The listing builds one solid part. Answer for the finished solid, in the listing's coordinates (mm). A direction names the side the tool comes from. Round coordinates to 2 decimals unless told otherwise and drop trailing zeros. Loops run counter-clockwise (first coordinate to the right, second up) from the corner with the lowest first, then second, coordinate; pieces in that order, holes last. Notation, with made-up numbers: (8.5, -23) - (38.5, -23) arc R32 cw to (38.5, 15) - close; hole circle Ø11 at (-31.5, 44). An arc over 180 degrees is marked (long way). One line per item, written item: value.
```python
from build123d import *

# Parameters (mm, degrees)
FLANGE_SKETCH_R              = 30
FRONT_FLANGE_60_DEPTH        = 16
FRONT_MAIN_JOURNAL_PROFILE_W = 15
FRONT_MAIN_JOURNAL_PROFILE_H = 62
CRANK_WEB_1_DEPTH            = 22
CRANKPIN_1_PROFILE_W         = 20
CRANKPIN_1_PROFILE_H         = 35
CRANK_WEB_2_DEPTH            = 25
MAIN_JOURNAL_2_PROFILE_W     = 22.5
MAIN_JOURNAL_2_PROFILE_H     = 35
CRANK_WEB_3_DEPTH            = 22
CRANKPIN_2_PROFILE_W         = 25
CRANKPIN_2_PROFILE_H         = 45
CRANK_WEB_4_DEPTH            = 25
MAIN_JOURNAL_3_PROFILE_W     = 22.5
MAIN_JOURNAL_3_PROFILE_H     = 46
CRANK_WEB_5_DEPTH            = 22
CRANKPIN_3_PROFILE_W         = 20
CRANKPIN_3_PROFILE_H         = 35
CRANK_WEB_6_SKETCH_R         = 20
CRANK_WEB_6_DEPTH            = 22
REAR_MAIN_JOURNAL_PROFILE_W  = 22.5
REAR_MAIN_JOURNAL_PROFILE_H  = 46
OUTPUT_SHAFT_PROFILE_W       = 25
OUTPUT_SHAFT_PROFILE_H       = 100
END_SPIGOT_PROFILE_W         = 12.5
END_SPIGOT_PROFILE_H         = 20
FLANGE_BOLT_HOLES_SKETCH_R   = 6
FLANGE_BOLT_HOLES_4X_DEPTH   = 22
FLANGE_CENTRE_RECESS_DEPTH   = 10


with BuildPart() as part:
    # Flange Sketch → Front Flange _60 (new body)
    with BuildSketch(Plane.XY):
        Circle(FLANGE_SKETCH_R)
    extrude(amount=FRONT_FLANGE_60_DEPTH)

    # Front Main Journal Profile → Front Main Journal (revolve)
    with BuildSketch(Plane(origin=(0, 0, 0), x_dir=(1, 0, 0), z_dir=(0, 1, 0)), mode=Mode.PRIVATE) as front_main_journal_sk:
        with Locations((7.5, 31)):
            Rectangle(FRONT_MAIN_JOURNAL_PROFILE_W, FRONT_MAIN_JOURNAL_PROFILE_H)
    revolve(front_main_journal_sk.sketch.rotate(Axis((0, 0, -63.530762812), (0, 0, 1)), 180), axis=Axis((0, 0, -63.530762812), (0, 0, 1)))

    # Crank Web 1 Sketch → Crank Web 1 (add)
    with BuildSketch(Plane(origin=(0, 0, -62), x_dir=(-1, 0, 0), z_dir=(0, 0, -1))):
        with BuildLine():
            Line((-40, 27.5), (0, 27.5))
            ThreePointArc((0, 27.5), (27.5, 0), (0, -27.5))
            Line((0, -27.5), (-40, -27.5))
            ThreePointArc((-40, -27.5), (-67.5, 0), (-40, 27.5))
        make_face()
    extrude(amount=CRANK_WEB_1_DEPTH)

    # Crankpin 1 Profile → Crankpin 1 (revolve)
    with BuildSketch(Plane(origin=(0, 0, 0), x_dir=(1, 0, 0), z_dir=(0, 1, 0))):
        with Locations((50, 101.5)):
            Rectangle(CRANKPIN_1_PROFILE_W, CRANKPIN_1_PROFILE_H)
    revolve(axis=Axis((40, 0, -84), (0, 0, -1)))

    # Crank Web 2 Sketch → Crank Web 2 (add)
    with BuildSketch(Plane(origin=(0, 0, -119), x_dir=(-1, 0, 0), z_dir=(0, 0, -1))):
        with BuildLine():
            Line((-40, 27.5), (40, 27.5))
            ThreePointArc((40, 27.5), (67.5, 0), (40, -27.5))
            Line((40, -27.5), (-40, -27.5))
            ThreePointArc((-40, -27.5), (-67.5, 0), (-40, 27.5))
        make_face()
    extrude(amount=CRANK_WEB_2_DEPTH)

    # Main Journal 2 Profile → Main Journal 2 (revolve)
    with BuildSketch(Plane(origin=(0, 0, 0), x_dir=(1, 0, 0), z_dir=(0, 1, 0))):
        with Locations((-28.75, 161.5)):
            Rectangle(MAIN_JOURNAL_2_PROFILE_W, MAIN_JOURNAL_2_PROFILE_H)
    revolve(axis=Axis((-40, 0, -144), (0, 0, -1)))

    # Crank Web 3 Sketch → Crank Web 3 (add)
    with BuildSketch(Plane(origin=(0, 0, -179), x_dir=(-1, 0, 0), z_dir=(0, 0, -1))):
        with BuildLine():
            Line((0, 27.5), (40, 27.5))
            ThreePointArc((40, 27.5), (67.5, 0), (40, -27.5))
            Line((40, -27.5), (0, -27.5))
            ThreePointArc((0, -27.5), (-27.5, 0), (0, 27.5))
        make_face()
    extrude(amount=CRANK_WEB_3_DEPTH)

    # Crankpin 2 Profile → Crankpin 2 (revolve)
    with BuildSketch(Plane(origin=(0, 0, 0), x_dir=(1, 0, 0), z_dir=(0, 1, 0)), mode=Mode.PRIVATE) as crankpin_2_sk:
        with Locations((12.5, 223.5)):
            Rectangle(CRANKPIN_2_PROFILE_W, CRANKPIN_2_PROFILE_H)
    revolve(crankpin_2_sk.sketch.rotate(Axis((0, 0, -261.148585065), (0, 0, 1)), 180), axis=Axis((0, 0, -261.148585065), (0, 0, 1)))

    # Crank Web 4 Sketch → Crank Web 4 (add)
    with BuildSketch(Plane(origin=(0, 0, -246), x_dir=(-1, 0, 0), z_dir=(0, 0, -1))):
        with BuildLine():
            Line((0, 27.5), (40, 27.5))
            ThreePointArc((40, 27.5), (67.5, 0), (40, -27.5))
            Line((40, -27.5), (0, -27.5))
            ThreePointArc((0, -27.5), (-27.5, 0), (0, 27.5))
        make_face()
    extrude(amount=CRANK_WEB_4_DEPTH)

    # Main Journal 3 Profile → Main Journal 3 (revolve)
    with BuildSketch(Plane(origin=(0, 0, 0), x_dir=(1, 0, 0), z_dir=(0, 1, 0))):
        with Locations((-28.75, 294)):
            Rectangle(MAIN_JOURNAL_3_PROFILE_W, MAIN_JOURNAL_3_PROFILE_H)
    revolve(axis=Axis((-40, 0, -271), (0, 0, -1)))

    # Crank Web 5 Sketch → Crank Web 5 (add)
    with BuildSketch(Plane(origin=(0, 0, -317), x_dir=(-1, 0, 0), z_dir=(0, 0, -1))):
        with BuildLine():
            Line((-40, 27.5), (40, 27.5))
            ThreePointArc((40, 27.5), (67.5, 0), (40, -27.5))
            Line((40, -27.5), (-40, -27.5))
            ThreePointArc((-40, -27.5), (-67.5, 0), (-40, 27.5))
        make_face()
    extrude(amount=CRANK_WEB_5_DEPTH)

    # Crankpin 3 Profile → Crankpin 3 (revolve)
    with BuildSketch(Plane(origin=(0, 0, 0), x_dir=(1, 0, 0), z_dir=(0, 1, 0))):
        with Locations((50, 356.5)):
            Rectangle(CRANKPIN_3_PROFILE_W, CRANKPIN_3_PROFILE_H)
    revolve(axis=Axis((40, 0, -339), (0, 0, -1)))

    # Crank Web 6 Sketch → Crank Web 6 (add)
    # profile 1 of 2: a face of its own
    with BuildSketch(Plane(origin=(0, 0, -374), x_dir=(-1, 0, 0), z_dir=(0, 0, -1))):
        with BuildLine():
            Line((-40, -27.5), (0, -27.5))
            ThreePointArc((0, -27.5), (27.5, 0), (0, 27.5))
            Line((0, 27.5), (-40, 27.5))
            ThreePointArc((-40, 27.5), (-67.5, 0), (-40, -27.5))
        make_face()
        with Locations(Location((-40, 0, 0), (0, 0, 180))):
            Circle(CRANK_WEB_6_SKETCH_R, mode=Mode.SUBTRACT)
    # profile 2 of 2: a face of its own
    with BuildSketch(Plane(origin=(0, 0, -374), x_dir=(-1, 0, 0), z_dir=(0, 0, -1))):
        with Locations(Location((-40, 0, 0), (0, 0, 180))):
            Circle(CRANK_WEB_6_SKETCH_R)
    extrude(amount=CRANK_WEB_6_DEPTH)

    # Rear Main Journal Profile → Rear Main Journal (revolve)
    with BuildSketch(Plane(origin=(0, 0, 0), x_dir=(1, 0, 0), z_dir=(0, 1, 0))):
        with Locations((11.25, 419)):
            Rectangle(REAR_MAIN_JOURNAL_PROFILE_W, REAR_MAIN_JOURNAL_PROFILE_H)
    revolve(axis=Axis((0, 0, -396), (0, 0, -1)))

    # Output Shaft Profile → Output Shaft (revolve)
    with BuildSketch(Plane(origin=(0, 0, 0), x_dir=(1, 0, 0), z_dir=(0, 1, 0))):
        with Locations((12.5, 492)):
            Rectangle(OUTPUT_SHAFT_PROFILE_W, OUTPUT_SHAFT_PROFILE_H)
    revolve(axis=Axis((0, 0, -442), (0, 0, -1)))

    # End Spigot Profile → End Spigot (revolve)
    with BuildSketch(Plane(origin=(0, 0, 0), x_dir=(1, 0, 0), z_dir=(0, 1, 0))):
        with Locations((6.25, 552)):
            Rectangle(END_SPIGOT_PROFILE_W, END_SPIGOT_PROFILE_H)
    revolve(axis=Axis((0, 0, -542), (0, 0, -1)))

    # Flange Bolt Holes Sketch → Flange Bolt Holes 4x (cut)
    with BuildSketch(Plane.XY.offset(16)):
        with Locations((22, 0)):
            Circle(FLANGE_BOLT_HOLES_SKETCH_R)
        with Locations((0.74374517, -21.25625483)):
            Circle(FLANGE_BOLT_HOLES_SKETCH_R)
        with Locations((-20.512509661, 0)):
            Circle(FLANGE_BOLT_HOLES_SKETCH_R)
        with Locations((0.74374517, 21.25625483)):
            Circle(FLANGE_BOLT_HOLES_SKETCH_R)
    extrude(amount=-FLANGE_BOLT_HOLES_4X_DEPTH, mode=Mode.SUBTRACT)

    # Flange Centre Recess Sketch → Flange Centre Recess (cut)
    with BuildSketch(Plane.XY.offset(16)):
        with BuildLine():
            Line((-10.897247359, 1.5), (-7.897247359, 1.5))
            Line((-7.897247359, 1.5), (-7.897247359, -1.5))
            Line((-7.897247359, -1.5), (-10.897247359, -1.5))
            ThreePointArc((-10.897247359, -1.5), (11, 0), (-10.897247359, 1.5))
        make_face()
    extrude(amount=-FLANGE_CENTRE_RECESS_DEPTH, mode=Mode.SUBTRACT)


solid = part.part
```
1) A cutting plane is placed at C-C on x = -57. Give the vertices of the cut face in (y, z).
Final values:
outline: (-21.62, -339) - (21.62, -339) - (21.62, -317) - (14.74, -317) - (14.74, -271) - (21.62, -271) - (21.62, -246) - (-21.62, -246) - (-21.62, -271) - (-14.74, -271) - (-14.74, -317) - (-21.62, -317) - close; (-21.62, -201) - (21.62, -201) - (21.62, -179) - (14.74, -179) - (14.74, -144) - (21.62, -144) - (21.62, -119) - (-21.62, -119) - (-21.62, -144) - (-14.74, -144) - (-14.74, -179) - (-21.62, -179) - close
2) A cutting plane is placed at D-D on z = -75. Give the vertices of the cut face in (x, y), and give its area (3 significant figures).
Final values:
outline: (0, -27.5) - (40, -27.5) arc R27.5 ccw to (40, 27.5) - (0, 27.5) arc R27.5 ccw to start
area: 4,580 mm2
3) A cutting plane is placed at B-B on z = -486. Give the vertices of the cut face in (x, y).
Final values:
outline: circle Ø50 at (0, 0)
4) Each of these flat-tipped pins is pushed along its axis until it touches: pin 1 Ø24 at (x, z) = (-10.5, -192.5) entering from -Y; pin 2 Ø4 at (x, y) = (-36, 18) entering from -Z; pin 3 Ø10 at (y, z) = (7, -331.5) entering from +X. Where does it stop, or does it pass through?
Final values:
pin 1: y = -27.5
pin 2: z = -339
pin 3: x = 67.43
5) For a pull along Z with two mould halves and no side action, classify faces 4 (the cylindrical face through (-29.618, 19.961, -294.322)), 5 (the flat face through (-14, -6, 0)), 6 (the flat face through (-20, -27.5, -190)) as released by +Z, released by -Z, zero draft, split by the parting line, or undercut.
Final values:
face 4: undercut
face 5: undercut
face 6: zero draft
6) Consider L1, parallel to Z at x = -2, y = 20; L2, parallel to Y at x = 0, z = 9; L3, parallel to Z at x = -5, y = 17. Determine where each line is inside the solid, lowest interval first.
Final values:
L1: -542 to -374, -339 to -317, -271 to -179, -144 to -119, -84 to -62
L2: -30 to -27.21, -15.3 to -11, 11 to 15.3, 27.21 to 30
L3: -542 to -374, -339 to -317, -271 to -179, -144 to -119, -84 to -62, 0 to 16
7) A cutting plane is placed at A-A on x = 50.5. Give the vertices of the cut face in (y, z), and give its area (3 significant figures).
Final values:
outline: (-25.42, -396) - (25.42, -396) - (25.42, -374) - (17.02, -374) - (17.02, -339) - (25.42, -339) - (25.42, -317) - (-25.42, -317) - (-25.42, -339) - (-17.02, -339) - (-17.02, -374) - (-25.42, -374) - close; (-25.42, -144) - (25.42, -144) - (25.42, -119) - (17.02, -119) - (17.02, -84) - (25.42, -84) - (25.42, -62) - (-25.42, -62) - (-25.42, -84) - (-17.02, -84) - (-17.02, -119) - (-25.42, -119) - close
area: 7,010 mm2
8) For faces 1 (the cylindrical face through (-29.97, 1.32, 7.89)), 2 (the cylindrical face through (59.076, -6.007, -356.745)), 3 (the flat face through (-20, -27.5, -258)), determine the directions among +Z, -Z, +X, -X, +Y, -Y from which every point of the face is accessible in a straight line to the end or side of a thin tool.
Final values:
face 1: +Z
face 2: none
face 3: -Z, +X, -X, -Y
